Part model, mm, in its own coordinate system. Round coordinates to 2 decimals unless told otherwise and drop trailing zeros. Write each loop counter-clockwise with the first axis right and the second up, starting at its lowest first coordinate (ties: lowest second). Pieces come first, ordered by that corner, then holes.
from build123d import *

# Parameters (mm, degrees)
BOSS_EXTRUDE1_DEPTH = 10


with BuildPart() as part:
    # Sketch1 → Boss-Extrude1 (new body)
    with BuildSketch(Plane.XY):
        Polygon((0, 0), (-340, 0), (-340, -225), (-310, -255), (0, -255), align=None)
        with BuildLine():
            Line((-293.5, -25), (-293.5, -75))
            ThreePointArc((-293.5, -75), (-300, -81.5), (-306.5, -75))
            Line((-306.5, -75), (-306.5, -25))
            ThreePointArc((-306.5, -25), (-300, -18.5), (-293.5, -25))
        make_face(mode=Mode.SUBTRACT)
        with BuildLine():
            Line((-153.5, -25), (-153.5, -75))
            ThreePointArc((-153.5, -75), (-160, -81.5), (-166.5, -75))
            Line((-166.5, -75), (-166.5, -25))
            ThreePointArc((-166.5, -25), (-160, -18.5), (-153.5, -25))
        make_face(mode=Mode.SUBTRACT)
        with BuildLine():
            Line((-293.5, -185), (-293.5, -235))
            ThreePointArc((-293.5, -235), (-300, -241.5), (-306.5, -235))
            Line((-306.5, -235), (-306.5, -185))
            ThreePointArc((-306.5, -185), (-300, -178.5), (-293.5, -185))
        make_face(mode=Mode.SUBTRACT)
        with BuildLine():
            Line((-153.5, -185), (-153.5, -235))
            ThreePointArc((-153.5, -235), (-160, -241.5), (-166.5, -235))
            Line((-166.5, -235), (-166.5, -185))
            ThreePointArc((-166.5, -185), (-160, -178.5), (-153.5, -185))
        make_face(mode=Mode.SUBTRACT)
    extrude(amount=-BOSS_EXTRUDE1_DEPTH)


solid = part.part
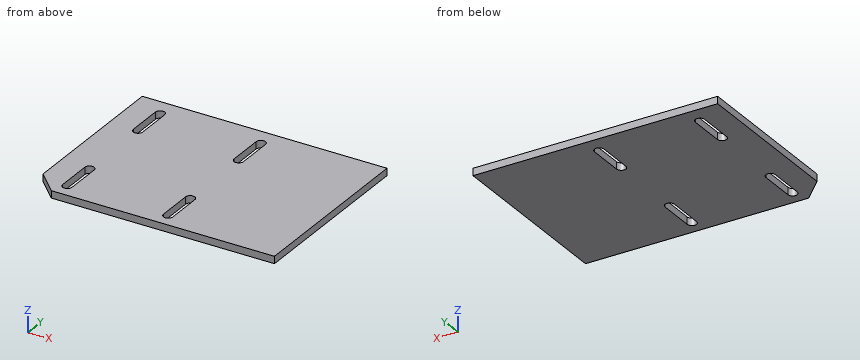
Q1. Saw through at B-B, the plane z = -4.5. Write the cut outline in (x, y).
Q2. Drop a flat-ended pin along its axis: P1, Ø5, axis at y = -60.5, z = -4.5, coming from the +X side. Give the stop position or say it passes through.
Q3. Wall check: line 1 (X direction, y = -31.5, z = -4); line 2 (X direction, y = -78.5, z = -2.5); line 3 (Y direction, x = -299, z = -1.5). Give the ranges that are in metal, low to high.
Q4. Saw through at A-A, the plane x = -300. Write the cut outline in (y, z), and give its area (3 significant figures).
Computed:
1. outline: (-340, -225) - (-310, -255) - (0, -255) - (0, 0) - (-340, 0) - close; hole (-306.5, -235) arc R6.5 ccw to (-293.5, -235) - (-293.5, -185) arc R6.5 ccw to (-306.5, -185) - close; hole (-306.5, -75) arc R6.5 ccw to (-293.5, -75) - (-293.5, -25) arc R6.5 ccw to (-306.5, -25) - close; hole (-166.5, -235) arc R6.5 ccw to (-153.5, -235) - (-153.5, -185) arc R6.5 ccw to (-166.5, -185) - close; hole (-166.5, -75) arc R6.5 ccw to (-153.5, -75) - (-153.5, -25) arc R6.5 ccw to (-166.5, -25) - close
2. P1: stops at x = 0
3. line 1: x = -340 to -306.5, -293.5 to -166.5, -153.5 to 0
3. line 2: x = -340 to -305.48, -294.52 to -165.48, -154.52 to 0
3. line 3: y = -255 to -241.42, -178.58 to -81.42, -18.58 to 0
4. outline: (-255, -10) - (-241.5, -10) - (-241.5, 0) - (-255, 0) - close; (-178.5, -10) - (-81.5, -10) - (-81.5, 0) - (-178.5, 0) - close; (-18.5, -10) - (0, -10) - (0, 0) - (-18.5, 0) - close
4. area: 1,290 mm2
